CAD build for the part. Positions are in the model's coordinates, mm. Face numbers are marked on the shaded views. Give positions to 0.01 mm unless a question says otherwise; leave off trailing zeros. Loops run counter-clockwise (first coordinate to the right, second up) from the corner with the lowest first, then second, coordinate; pieces in that order, holes last.
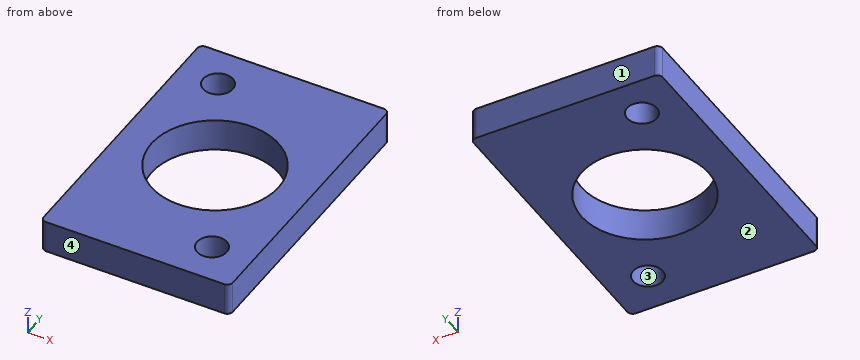
```python
from build123d import *

# Parameters (mm, degrees)
SKETCH_1_R      = 23.5
SKETCH_1_R_2    = 5.5
EXTRUDE_1_DEPTH = 12


with BuildPart() as part:
    # 草图1 → 凸台-拉伸1 (new body)
    with BuildSketch(Plane.XY):
        with BuildLine():
            Line((-33, 52.5), (33, 52.5))
            ThreePointArc((33, 52.5), (34.414213562, 51.914213562), (35, 50.5))
            Line((35, 50.5), (35, -50.5))
            ThreePointArc((35, -50.5), (34.414213562, -51.914213562), (33, -52.5))
            Line((33, -52.5), (-33, -52.5))
            ThreePointArc((-33, -52.5), (-34.414213562, -51.914213562), (-35, -50.5))
            Line((-35, -50.5), (-35, 50.5))
            ThreePointArc((-35, 50.5), (-34.414213562, 51.914213562), (-33, 52.5))
        make_face()
        Circle(SKETCH_1_R, mode=Mode.SUBTRACT)
        with Locations((-20, 37.5)):
            Circle(SKETCH_1_R_2, mode=Mode.SUBTRACT)
        with Locations((20, -37.5)):
            Circle(SKETCH_1_R_2, mode=Mode.SUBTRACT)
    extrude(amount=EXTRUDE_1_DEPTH)


solid = part.part
```
1. Probe line 1 along Y through (x, z) = (20, 4); line 2 along Y through (x, z) = (-20, 5.25); line 3 along X through (y, z) = (0.5, 10.25). List the from-to ranges inside material, lowest first.
Responses:
line 1: y = -52.5 to -43, -32 to -12.34, 12.34 to 52.5
line 2: y = -52.5 to -12.34, 12.34 to 32, 43 to 52.5
line 3: x = -35 to -23.49, 23.49 to 35
2. Saw through at D-D, the plane x = 20. List the corners of the cut face in (y, z), and give its area (3 significant figures).
Responses:
outline: (-52.5, 0) - (-43, 0) - (-43, 12) - (-52.5, 12) - close; (-32, 0) - (-12.34, 0) - (-12.34, 12) - (-32, 12) - close; (12.34, 0) - (52.5, 0) - (52.5, 12) - (12.34, 12) - close
area: 832 mm2
3. Saw through at C-C, the plane z = 8.25. List the corners of the cut face in (x, y), and give its area (3 significant figures).
Responses:
outline: (-35, -50.5) arc R2 ccw to (-33, -52.5) - (33, -52.5) arc R2 ccw to (35, -50.5) - (35, 50.5) arc R2 ccw to (33, 52.5) - (-33, 52.5) arc R2 ccw to (-35, 50.5) - close; hole circle Ø11 at (-20, 37.5); hole circle Ø47 at (0, 0); hole circle Ø11 at (20, -37.5)
area: 5,420 mm2
4. Saw through at A-A, the plane y = 37.5. List the corners of the cut face in (x, z).
Responses:
outline: (-35, 0) - (-25.5, 0) - (-25.5, 12) - (-35, 12) - close; (-14.5, 0) - (35, 0) - (35, 12) - (-14.5, 12) - close
5. Drop a flat-ended pin along its axis: pin 1 (6.5 mm diameter, centred on x = -20, y = 37.5, fed in from -Z). Give the stop position or say it passes through.
Responses:
pin 1: passes through
6. Saw through at B-B, the plane x = 0. List the corners of the cut face in (y, z), and give its area (3 significant figures).
Responses:
outline: (-52.5, 0) - (-23.5, 0) - (-23.5, 12) - (-52.5, 12) - close; (23.5, 0) - (52.5, 0) - (52.5, 12) - (23.5, 12) - close
area: 696 mm2
7. Pull direction Y, two halves, no side cores. Call the marked faces 1, 2, 3 and 4: released by +Y, released by -Y, zero draft, split by the parting line, or undercut.
Responses:
face 1: released by +Y
face 2: zero draft
face 3: undercut
face 4: released by -Y
